Read the model definition and answer for the solid it produces. Units are mm, in the model's axes. A direction names the side the tool comes from. Coordinates: 2 decimals unless noted, no trailing zeros. Loops run counter-clockwise (first coordinate to the right, second up) from the corner with the lowest first, then second, coordinate; pieces in that order, holes last. Notation, with made-up numbers: (26.25, -30) -> (35.25, -30) arc R17 ccw to (35.25, -22) -> close; hole circle Ø8 at (-39.5, -24). An arc over 180 degrees is marked (long way). Answer as a JSON object with one key per item and string values. Group by question number.
Q1. The part is cut by section B-B on x = -5. Write down the section's boundary in (y, z).
Q2. The part is cut by section A-A on z = 0. Write down the section's boundary in (x, y), and give its area (3 significant figures).
Q3. Each of these flat-tipped pins is pushed along its axis until it touches: P1, Ø4, axis at x = 3, z = -23.5, coming from the +Y side; P2, Ø5, axis at x = 11, z = -13, coming from the +Y side; P3, Ø2, axis at x = 3, y = 27, coming from the -Z side. Where does it stop, or does it pass through?
Q4. The part is cut by section C-C on y = 43. Write down the section's boundary in (x, z), and give its area (3 significant figures).
Q5. The part is cut by section D-D on y = 52. Write down the section's boundary in (x, z), and give its area (3 significant figures).
Q6. Determine the mould class of faces 1 (the flat face through (13, 56.5, 0)), 2 (the flat face through (15, 23, 1)), 3 (the flat face through (0, 5, -45)) for opening direction Y: released by +Y, released by -Y, zero draft, split by the parting line, or undercut.
Q7. Straight lines are drawn through the part: line 1 along Y through (x, z) = (9.5, 0); line 2 along X through (y, z) = (43.5, -15); line 3 along X through (y, z) = (46, 21.5). For each, find the intervals that lie inside material, in ascending order. Write a range as [from, to].
Q8. For faces 4 (the flat face through (0, 39.5, -20)), 5 (the flat face through (-25, 5, 1)), 6 (the cylindrical face through (22.605, 26.892, 3.577)), 7 (the flat face through (20, 10, -1)), determine the directions among +Z, -Z, +X, -X, +Y, -Y from which every point of the face is accessible in a straight line to the end or side of a thin tool.
from build123d import *

# Parameters (mm, degrees)
BASE_PLATE_SKETCH_W        = 50
BASE_PLATE_SKETCH_H        = 90
BASE_PLATE_90X50X10_DEPTH  = 10
UPRIGHT_PROFILE_SKETCH_W   = 30
UPRIGHT_PROFILE_SKETCH_H   = 90
TAPERED_UPRIGHT_DEPTH      = 56.5
UPRIGHT_TRIM_SKETCH_W      = 14
UPRIGHT_TRIM_SKETCH_H      = 27
UPRIGHT_TRIM_CUT_DEPTH     = 115.661458215
BEARING_BOSS_SKETCH_R      = 16.5
BEARING_BOSS_SKETCH_R_2    = 6
BEARING_BOSS_DEPTH         = 30
CENTRE_SLOT_SKETCH_W       = 46
CENTRE_SLOT_SKETCH_H       = 10
CENTRE_SLOT_CUT_DEPTH      = 65
TOP_SLOT_CUT_DEPTH         = 65
BEARING_BORE_SKETCH_R      = 6
BEARING_BORE_THROUGH_DEPTH = 65
BOSS_NOTCH_SKETCH_W        = 14
BOSS_NOTCH_SKETCH_H        = 17
BOSS_NOTCH_CUT_DEPTH       = 65


with BuildPart() as part:
    # Base Plate Sketch → Base Plate 90x50x10 (new body)
    with BuildSketch(Plane(origin=(0, 0, 0), x_dir=(1, 0, 0), z_dir=(0, 1, 0))):
        Rectangle(BASE_PLATE_SKETCH_W, BASE_PLATE_SKETCH_H)
    extrude(amount=BASE_PLATE_90X50X10_DEPTH)

    # Upright Profile Sketch → Tapered Upright (add)
    with BuildSketch(Plane(origin=(0, 10, 0), x_dir=(1, 0, 0), z_dir=(0, 1, 0))):
        Rectangle(UPRIGHT_PROFILE_SKETCH_W, UPRIGHT_PROFILE_SKETCH_H)
    extrude(amount=TAPERED_UPRIGHT_DEPTH)

    # Upright Trim Sketch → Upright Trim Cut (cut, through all)
    with BuildSketch(Plane.XY.offset(45)):
        with Locations((0, 53)):
            Rectangle(UPRIGHT_TRIM_SKETCH_W, UPRIGHT_TRIM_SKETCH_H)
    extrude(amount=-UPRIGHT_TRIM_CUT_DEPTH, mode=Mode.SUBTRACT)

    # Bearing Boss Sketch → Bearing Boss (add, symmetric)
    with BuildSketch(Plane(origin=(0, 0, 0), x_dir=(0, 0, -1), z_dir=(1, 0, 0))):
        with Locations((0, 43)):
            Circle(BEARING_BOSS_SKETCH_R)
        with Locations((0, 43)):
            Circle(BEARING_BOSS_SKETCH_R_2, mode=Mode.SUBTRACT)
    extrude(amount=BEARING_BOSS_DEPTH, both=True)

    # Centre Slot Sketch → Centre Slot Cut (cut, symmetric)
    with BuildSketch(Plane.XY):
        with Locations((0, 61.5)):
            Rectangle(CENTRE_SLOT_SKETCH_W, CENTRE_SLOT_SKETCH_H)
    extrude(amount=CENTRE_SLOT_CUT_DEPTH, both=True, mode=Mode.SUBTRACT)

    # Top Slot Sketch → Top Slot Cut (cut, symmetric)
    with BuildSketch(Plane(origin=(0, 0, 0), x_dir=(0, 0, -1), z_dir=(1, 0, 0))):
        Polygon((-31.5, 56.5), (-45, 10), (-45, 56.5), align=None)
        Polygon((31.5, 56.5), (45, 10), (45, 56.5), align=None)
    extrude(amount=TOP_SLOT_CUT_DEPTH, both=True, mode=Mode.SUBTRACT)

    # Bearing Bore Sketch → Bearing Bore Through (cut, symmetric)
    with BuildSketch(Plane.ZY.offset(15)):
        with Locations(Location((0, 43, 0), (0, 0, 180))):
            Circle(BEARING_BORE_SKETCH_R)
    extrude(amount=BEARING_BORE_THROUGH_DEPTH, both=True, mode=Mode.SUBTRACT)

    # Boss Notch Sketch → Boss Notch Cut (cut, symmetric)
    with BuildSketch(Plane.XY):
        with Locations((0, 48)):
            Rectangle(BOSS_NOTCH_SKETCH_W, BOSS_NOTCH_SKETCH_H)
    extrude(amount=BOSS_NOTCH_CUT_DEPTH, both=True, mode=Mode.SUBTRACT)


solid = part.part
Final values:
{
 "1": {"outline": "(0, -45) -> (10, -45) -> (39.5, -36.44) -> (39.5, -4.87) arc R6 cw to (39.5, 4.87) -> (39.5, 36.44) -> (10, 45) -> (0, 45) -> close"},
 "2": {"outline": "(-30, 26.5) -> (-15, 26.5) -> (-15, 10) -> (-25, 10) -> (-25, 0) -> (25, 0) -> (25, 10) -> (15, 10) -> (15, 26.5) -> (30, 26.5) -> (30, 37) -> (-30, 37) -> close; (-30, 49) -> (-7, 49) -> (-7, 56.5) -> (-23, 56.5) -> (-23, 59.5) -> (-30, 59.5) -> close; (7, 49) -> (30, 49) -> (30, 59.5) -> (23, 59.5) -> (23, 56.5) -> (7, 56.5) -> close", "area": "2,010 mm2"},
 "3": {"P1": "stops at y = 39.5", "P2": "stops at y = 56.5", "P3": "stops at z = -40.35"},
 "4": {"outline": "(-30, -16.5) -> (-15, -16.5) -> (-15, -35.42) -> (-7, -35.42) -> (-7, -6) -> (-30, -6) -> close; (-30, 6) -> (-7, 6) -> (-7, 35.42) -> (-15, 35.42) -> (-15, 16.5) -> (-30, 16.5) -> close; (7, -35.42) -> (15, -35.42) -> (15, -16.5) -> (30, -16.5) -> (30, -6) -> (7, -6) -> close; (7, 6) -> (30, 6) -> (30, 16.5) -> (15, 16.5) -> (15, 35.42) -> (7, 35.42) -> close", "area": "1,570 mm2"},
 "5": {"outline": "(-30, -13.83) -> (-15, -13.83) -> (-15, -32.81) -> (-7, -32.81) -> (-7, 32.81) -> (-15, 32.81) -> (-15, 13.83) -> (-30, 13.83) -> close; (7, -32.81) -> (15, -32.81) -> (15, -13.83) -> (30, -13.83) -> (30, 13.83) -> (15, 13.83) -> (15, 32.81) -> (7, 32.81) -> close", "area": "1,880 mm2"},
 "6": {"face 1": "released by +Y", "face 2": "undercut", "face 3": "zero draft"},
 "7": {"line 1": "y = [0, 37], [49, 56.5]", "line 2": "x = [-30, -7], [7, 30]", "line 3": "x = [-15, -7], [7, 15]"},
 "8": {"face 4": "+Z, -Z, +Y", "face 5": "+Z, -Z, -X, -Y", "face 6": "+X", "face 7": "+Z, -Z, +X"}
}
